from build123d import *

# Parameters (mm, degrees)
BOSS_EXTRUDE1_DEPTH          = 2.5
SKETCH2_W                    = 90
SKETCH2_H                    = 2.5
BOSS_EXTRUDE2_DEPTH          = 40.000031182
BOSS_EXTRUDE3_DEPTH          = 2.5
F_6_0_6_DIAMETER_HOLE1_D     = 6
F_6_0_6_DIAMETER_HOLE1_DEPTH = 2.5
F_6_0_6_DIAMETER_HOLE2_D     = 6
F_6_0_6_DIAMETER_HOLE2_DEPTH = 2.5
F_10_0_10_DIAMETER_HOLE1_D   = 10
F_6_0_6_DIAMETER_HOLE3_D     = 6
FILLET1_R                    = 0.7366
FILLET2_R                    = 3.2366


with BuildPart() as part:
    # Sketch1 → Boss-Extrude1 (new body)
    with BuildSketch(Plane(origin=(-22.498134156, 0, 0), x_dir=(0, -1, 0), z_dir=(-1, 0, 0))):
        with BuildLine():
            Line((-5.354521861, -90), (2.5, -90))
            Line((2.5, -90), (2.5, 0))
            Line((2.5, 0), (-5.354521861, 0))
            ThreePointArc((-5.354521861, 0), (-12.354521861, -7), (-5.354521861, -14))
            Line((-5.354521861, -14), (-5.354521861, -41))
            Line((-5.354521861, -41), (-6.354521861, -41))
            ThreePointArc((-6.354521861, -41), (-9.05608398, -42.298437881), (-10.354521861, -45))
            ThreePointArc((-10.354521861, -45), (-9.05608398, -47.701562119), (-6.354521861, -49))
            Line((-6.354521861, -49), (-5.354521861, -49))
            Line((-5.354521861, -49), (-5.354521861, -76))
            ThreePointArc((-5.354521861, -76), (-12.354521861, -83), (-5.354521861, -90))
        make_face()
    extrude(amount=-BOSS_EXTRUDE1_DEPTH)

    # Sketch2 → Boss-Extrude2 (add)
    with BuildSketch(Plane(origin=(-19.998134156, 0, 0), x_dir=(0, 0, -1), z_dir=(1, 0, 0))):
        with Locations((45, -1.25)):
            Rectangle(SKETCH2_W, SKETCH2_H)
    extrude(amount=BOSS_EXTRUDE2_DEPTH)

    # Sketch3 → Boss-Extrude3 (add)
    with BuildSketch(Plane(origin=(20.001897026, 0, 0), x_dir=(0, 0, -1), z_dir=(1, 0, 0))):
        with BuildLine():
            Line((0, -2.5), (0, 5.350758991))
            ThreePointArc((0, 5.350758991), (7, 12.350758991), (14, 5.350758991))
            Line((14, 5.350758991), (41, 5.350758991))
            Line((41, 5.350758991), (41, 6.350758991))
            ThreePointArc((41, 6.350758991), (42.298437881, 9.05232111), (45, 10.350758991))
            ThreePointArc((45, 10.350758991), (47.701562119, 9.05232111), (49, 6.350758991))
            Line((49, 6.350758991), (49, 5.350758991))
            Line((49, 5.350758991), (76, 5.350758991))
            ThreePointArc((76, 5.350758991), (83, 12.350758991), (90, 5.350758991))
            Line((90, 5.350758991), (90, -2.5))
            Line((90, -2.5), (0, -2.5))
        make_face()
    extrude(amount=BOSS_EXTRUDE3_DEPTH)

    # Ø6.0 (6) Diameter Hole1
    with Locations(Plane.ZY.offset(-20.001897026)):
        with Locations((-83, 6.850758991), (-7, 6.350758991)):
            Hole(F_6_0_6_DIAMETER_HOLE1_D / 2, depth=F_6_0_6_DIAMETER_HOLE1_DEPTH)

    # Ø6.0 (6) Diameter Hole2
    with Locations(Plane(origin=(-19.998134156, 0, 0), x_dir=(0, 0, -1), z_dir=(1, 0, 0))):
        with Locations((83, 6.854521861), (7, 6.354521861)):
            Hole(F_6_0_6_DIAMETER_HOLE2_D / 2, depth=F_6_0_6_DIAMETER_HOLE2_DEPTH)

    # Ø10.0 (10) Diameter Hole1 (through all)
    with Locations(Plane(origin=(0, 0, 0), x_dir=(1, 0, 0), z_dir=(0, 1, 0))):
        with Locations((0, 45), (-10, 57), (-10, 33), (10, 33), (10, 57)):
            Hole(F_10_0_10_DIAMETER_HOLE1_D / 2)

    # Ø6.0 (6) Diameter Hole3 (through all)
    with Locations(Plane(origin=(0, 0, 0), x_dir=(1, 0, 0), z_dir=(0, 1, 0))):
        with Locations((0, 70), (0, 20)):
            Hole(F_6_0_6_DIAMETER_HOLE3_D / 2)

    # Fillet1
    fillet1_edges = [part.edges().sort_by_distance(p)[0] for p in [
        (-19.998134156, 0, -45),
        (20.001897026, 0, -45),
    ]]
    fillet(fillet1_edges, radius=FILLET1_R)

    # Fillet2
    fillet2_edges = [part.edges().sort_by_distance(p)[0] for p in [
        (-22.498134156, -2.5, -45),
        (22.501897026, -2.5, -45),
    ]]
    fillet(fillet2_edges, radius=FILLET2_R)


solid = part.part
Here's how the part is built. I have some questions about the finished solid (model axes, mm). A direction names the side the tool comes from. Coordinates: 2 decimals unless noted, no trailing zeros. Loops run counter-clockwise (first coordinate to the right, second up) from the corner with the lowest first, then second, coordinate; pieces in that order, holes last.
1. For faces 1 (the flat face through (21, 5.351, -62)), 2 (the cylindrical face through (21.579, -1.527, -44.37)), 3 (the flat face through (20.002, 4, -46)), which set-ups out of +Z, -Z, +X, -X, +Y, -Y let a thin tool reach every point of the face, with its end or its side?
2. If we mould it in two halves opening along Z, with no side actions, what happens to faces 4 (the flat face through (8, 0, -44)), 5 (the cylindrical face through (0.65, -1.27, -67.07)), 6 (the cylindrical face through (21.234, 9.082, -47.671))? For each: pulls with the +Z half, pulls with the -Z half, needs draft (parallel to the pull), parting line crosses it, or undercut.
3. I need wall thicknesses on L1, parallel to Z at x = 10, y = -1.95; L2, parallel to X at y = -0.45, z = -57; L3, parallel to X at y = 10, z = -79. Which ranges of each line are inside material? Lowest first, please.
4. For P1, Ø4, axis at x = -12.5, z = -33.5, coming from the +Y side; P2, Ø1.2, axis at x = 21.5, z = -57.5, coming from the +Y side; P3, Ø9.5, axis at x = 0, z = -20, coming from the +Y side; P4, Ø13, axis at x = -10, z = -33, coming from the -Y side, each with a flat end and sliding along its axis, tell me the tip position at first contact or that it passes through.
5. Imagine slicing it at C-C, the plane y = 2. Please give me the cut outline in (x, z).
6. Imagine slicing it at B-B, the plane z = -7. Please give me the cut outline in (x, y), and give its area (3 significant figures).
7. Imagine slicing it at A-A, the plane x = 0. Please give me the cut outline in (y, z).
8. Imagine slicing it at D-D, the plane x = 10. Please give me the cut outline in (y, z), and give its area (3 significant figures).
Taken from the geometry:
1. face 1: +X, -X, +Y
1. face 2: +Z, -Z, +X, -Y
1. face 3: +Z, -Z, +Y
2. face 4: needs draft
2. face 5: undercut
2. face 6: undercut
3. L1: z = -90 to -62, -52 to -38, -28 to 0
3. L2: x = -22.27 to -15, -5 to 5, 15 to 22.28
3. L3: x = -22.5 to -20, 20 to 22.5
4. P1: passes through
4. P2: stops at y = 5.35
4. P3: stops at y = 0
4. P4: stops at y = -2.5
5. outline: (-22.5, -90) - (-20, -90) - (-20, 0) - (-22.5, 0) - close; (20, -90) - (22.5, -90) - (22.5, 0) - (20, 0) - close
6. outline: (-22.5, 0.74) arc R3.24 ccw to (-19.26, -2.5) - (19.27, -2.5) arc R3.24 ccw to (22.5, 0.74) - (22.5, 3.35) - (20, 3.35) - (20, 0.74) arc R0.74 cw to (19.27, 0) - (-19.26, 0) arc R0.74 cw to (-20, 0.74) - (-20, 3.35) - (-22.5, 3.35) - close; (-22.5, 9.35) - (-20, 9.35) - (-20, 12.35) - (-22.5, 12.35) - close; (20, 9.35) - (22.5, 9.35) - (22.5, 12.35) - (20, 12.35) - close
6. area: 140 mm2
7. outline: (-2.5, -90) - (0, -90) - (0, -73) - (-2.5, -73) - close; (-2.5, -67) - (0, -67) - (0, -50) - (-2.5, -50) - close; (-2.5, -40) - (0, -40) - (0, -23) - (-2.5, -23) - close; (-2.5, -17) - (0, -17) - (0, 0) - (-2.5, 0) - close
8. outline: (-2.5, -90) - (0, -90) - (0, -62) - (-2.5, -62) - close; (-2.5, -52) - (0, -52) - (0, -38) - (-2.5, -38) - close; (-2.5, -28) - (0, -28) - (0, 0) - (-2.5, 0) - close
8. area: 175 mm2
